Verification items for the finished model (mm, model axes). Coordinates: 2 decimals unless noted, no trailing zeros. Write each loop counter-clockwise with the first axis right and the second up, starting at its lowest first coordinate (ties: lowest second). Pieces come first, ordered by that corner, then holes. Notation, with made-up numbers: M 39.5,-8 L 79.5,-8 A36 cw 79.5,30 Z; hole C 66.25,23 d9. An arc over 180 degrees is marked long. One line per item, written item: value.
```python
from build123d import *

# Parameters (mm, degrees)
SKETCH_1_R      = 1.3
EXTRUDE_1_DEPTH = 1.5
FILLET_1_R      = 2
FILLET_2_R      = 1
FILLET_3_R      = 20
FILLET_4_R      = 3


with BuildPart() as part:
    # 草图1 → 凸台-拉伸1 (new body)
    with BuildSketch(Plane.XY):
        with BuildLine():
            Line((-19.040408206, -33.5), (19.040408206, -33.5))
            ThreePointArc((19.040408206, -33.5), (20.181877211, -34.177811626), (21.507254803, -34.253668928))
            Line((21.507254803, -34.253668928), (40.507254803, -30.753668928))
            ThreePointArc((40.507254803, -30.753668928), (42.753668928, -27.492745197), (39.492745197, -25.246331072))
            Line((39.492745197, -25.246331072), (23, -28.284468345))
            Line((23, -28.284468345), (23, 28.284468345))
            Line((23, 28.284468345), (39.492745197, 25.246331072))
            ThreePointArc((39.492745197, 25.246331072), (42.753668928, 27.492745197), (40.507254803, 30.753668928))
            Line((40.507254803, 30.753668928), (21.507254803, 34.253668928))
            ThreePointArc((21.507254803, 34.253668928), (20.181877211, 34.177811626), (19.040408206, 33.5))
            Line((19.040408206, 33.5), (-19.040408206, 33.5))
            ThreePointArc((-19.040408206, 33.5), (-20.181877211, 34.177811626), (-21.507254803, 34.253668928))
            Line((-21.507254803, 34.253668928), (-40.507254803, 30.753668928))
            ThreePointArc((-40.507254803, 30.753668928), (-42.753668928, 27.492745197), (-39.492745197, 25.246331072))
            Line((-39.492745197, 25.246331072), (-23, 28.284468345))
            Line((-23, 28.284468345), (-23, -28.284468345))
            Line((-23, -28.284468345), (-39.492745197, -25.246331072))
            ThreePointArc((-39.492745197, -25.246331072), (-42.753668928, -27.492745197), (-40.507254803, -30.753668928))
            Line((-40.507254803, -30.753668928), (-21.507254803, -34.253668928))
            ThreePointArc((-21.507254803, -34.253668928), (-20.181877211, -34.177811626), (-19.040408206, -33.5))
        make_face()
        with Locations((-40, -28)):
            Circle(SKETCH_1_R, mode=Mode.SUBTRACT)
        with Locations((-21, -31.5)):
            Circle(SKETCH_1_R, mode=Mode.SUBTRACT)
        with Locations((40, -28)):
            Circle(SKETCH_1_R, mode=Mode.SUBTRACT)
        Polygon((0, -2.704163457), (17.863891029, -29.5), (-17.863891029, -29.5), align=None, mode=Mode.SUBTRACT)
        Polygon((-19, 25.795836543), (-1.802775638, 0), (-19, -25.795836543), align=None, mode=Mode.SUBTRACT)
        with Locations((-40, 28)):
            Circle(SKETCH_1_R, mode=Mode.SUBTRACT)
        with Locations((-21, 31.5)):
            Circle(SKETCH_1_R, mode=Mode.SUBTRACT)
        Polygon((19, -25.795836543), (1.802775638, 0), (19, 25.795836543), align=None, mode=Mode.SUBTRACT)
        Polygon((0, 2.704163457), (-17.863891029, 29.5), (17.863891029, 29.5), align=None, mode=Mode.SUBTRACT)
        with Locations((21, 31.5)):
            Circle(SKETCH_1_R, mode=Mode.SUBTRACT)
        with Locations((40, 28)):
            Circle(SKETCH_1_R, mode=Mode.SUBTRACT)
        with Locations((21, -31.5)):
            Circle(SKETCH_1_R, mode=Mode.SUBTRACT)
    extrude(amount=EXTRUDE_1_DEPTH)

    # 圆角1
    fillet_1_edges = [part.edges().sort_by_distance(p)[0] for p in [
        (17.863891029, -29.5, 0.75),
        (0, -2.704163457, 0.75),
        (-17.863891029, -29.5, 0.75),
        (-17.863891029, 29.5, 0.75),
        (0, 2.704163457, 0.75),
        (17.863891029, 29.5, 0.75),
    ]]
    fillet(fillet_1_edges, radius=FILLET_1_R)

    # 圆角2
    fillet_2_edges = [part.edges().sort_by_distance(p)[0] for p in [
        (19, -25.795836543, 0.75),
        (19, 25.795836543, 0.75),
        (-19, 25.795836543, 0.75),
        (-19, -25.795836543, 0.75),
    ]]
    fillet(fillet_2_edges, radius=FILLET_2_R)

    # 圆角3
    fillet_3_edges = [part.edges().sort_by_distance(p)[0] for p in [
        (19.040408206, 33.5, 0.75),
        (19.040408206, -33.5, 0.75),
        (-19.040408206, -33.5, 0.75),
        (-19.040408206, 33.5, 0.75),
    ]]
    fillet(fillet_3_edges, radius=FILLET_3_R)

    # 圆角4
    fillet_4_edges = [part.edges().sort_by_distance(p)[0] for p in [
        (1.802775638, 0, 0.75),
        (-1.802775638, 0, 0.75),
        (23, 28.284468345, 0.75),
        (23, -28.284468345, 0.75),
        (-23, -28.284468345, 0.75),
        (-23, 28.284468345, 0.75),
    ]]
    fillet(fillet_4_edges, radius=FILLET_4_R)


solid = part.part
```
Item 1: Cross-section at B-B, the plane x = 8. Enter the section's corners in (y, z), and give its area (3 significant figures).
The answers:
outline: M -33.5,0 L -29.5,0 L -29.5,1.5 L -33.5,1.5 Z; M -14.7,0 L -9.3,0 L -9.3,1.5 L -14.7,1.5 Z; M 9.3,0 L 14.7,0 L 14.7,1.5 L 9.3,1.5 Z; M 29.5,0 L 33.5,0 L 33.5,1.5 L 29.5,1.5 Z
area: 28.2 mm²
Item 2: Cross-section at C-C, the plane x = -34.5. Enter the section's corners in (y, z).
The answers:
outline: M -31.86,0 L -26.17,0 L -26.17,1.5 L -31.86,1.5 Z; M 26.17,0 L 31.86,0 L 31.86,1.5 L 26.17,1.5 Z
Item 3: Scan lines: line 1 (X direction, y = 2.5, z = 0.7); line 2 (X direction, y = 6.5, z = 0.5); line 3 (Y direction, x = 22, z = 1.3). Record each from-to range of solid material in increasing order.
The answers:
line 1: x = -23 to -19, -3.47 to 3.47, 19 to 23
line 2: x = -23 to -19, -6.14 to -2.53, 2.53 to 6.14, 19 to 23
line 3: y = -34.16 to -32.33, -30.67 to 30.67, 32.33 to 34.16
Item 4: Go/stop test with flat-tipped pins: P1, Ø0.8, axis at x = 6.5, z = 1, coming from the +Y side; P2, Ø0.8, axis at y = 0.5, z = 1, coming from the +X side. Record where each tip stops, or that it passes through.
The answers:
P1: stops at y = 33.5
P2: stops at x = 23
Item 5: Cross-section at A-A, the plane y = 15.5. Enter the section's corners in (x, z).
The answers:
outline: M -23,0 L -19,0 L -19,1.5 L -23,1.5 Z; M -12.14,0 L -8.53,0 L -8.53,1.5 L -12.14,1.5 Z; M 8.53,0 L 12.14,0 L 12.14,1.5 L 8.53,1.5 Z; M 19,0 L 23,0 L 23,1.5 L 19,1.5 Z
Item 6: Cross-section at D-D, the plane z = 1.1. Give the number of separate pieces and of enclosed holes in the cut face, and give its area (3 significant figures).
The answers:
separate pieces: 1
enclosed holes: 12
area: 1,680 mm²
Item 7: Draft check along X on faces 1 (the face through (30.87, -32.53, 0.74)), 2 (the face through (-21.958, -30.621, 0.74)), 3 (the face through (-1, 0, 0)), 4 (the face through (-10.14, 12.506, 0.74)). Enter one of: released by +X, released by -X, zero draft, split by the parting line, or undercut.
The answers:
face 1: released by +X
face 2: undercut
face 3: zero draft
face 4: undercut
